Design review of the part shown in the three views and the two pictorial views. Dimensions are in mm from the part's minimum x, y and z. A direction names the side the tool comes from. Round coordinates to 2 decimals unless told otherwise and drop trailing zeros. Loops run counter-clockwise (first coordinate to the right, second up) from the corner with the lowest first, then second, coordinate; pieces in that order, holes last.
1. Clearance check with flat-ended pins moving along their axes: pin 1 Ø17.5 at (x, y) = (31, 45) entering from +Z; pin 2 Ø12 at (x, z) = (50, 108) entering from +Y; pin 3 Ø3 at (x, z) = (20, 16.5) entering from +Y. State where each tip first meets the part, or that it passes through.
2. Tool access review of the marked faces 1, 2, 3 and 4: name each direction out of +Z, -Z, +X, -X, +Y, -Y from which nothing blocks a thin tool from reaching the whole face with its end or side.
3. To check wall thickness, follow line 1 along Y through (x, z) = (49.5, 134) (1 decimal); line 2 along Y through (x, z) = (37, 35.5); line 3 along Y through (x, z) = (48.5, 8.5). State the ranges of each line that lie inside material, in increasing order.
4. Consider section A-A on x = 34. State the section outline as (y, z) points, then the cut area to 3 significant figures.
5. Draft analysis for pull direction Z (two halves, no side actions). For the marked faces 5, 6 and 7, state which applies: released by +Z, released by -Z, zero draft, split by the parting line, or undercut.
6. Consider section C-C on z = 28. State the section outline as (x, y) points, then the cut area to 3 significant figures.
7. Consider section D-D on x = 54. State the section outline as (y, z) points, then the cut area to 3 significant figures.
8. Consider section B-B on y = 37.5. State the section outline as (x, z) points, then the cut area to 3 significant figures.
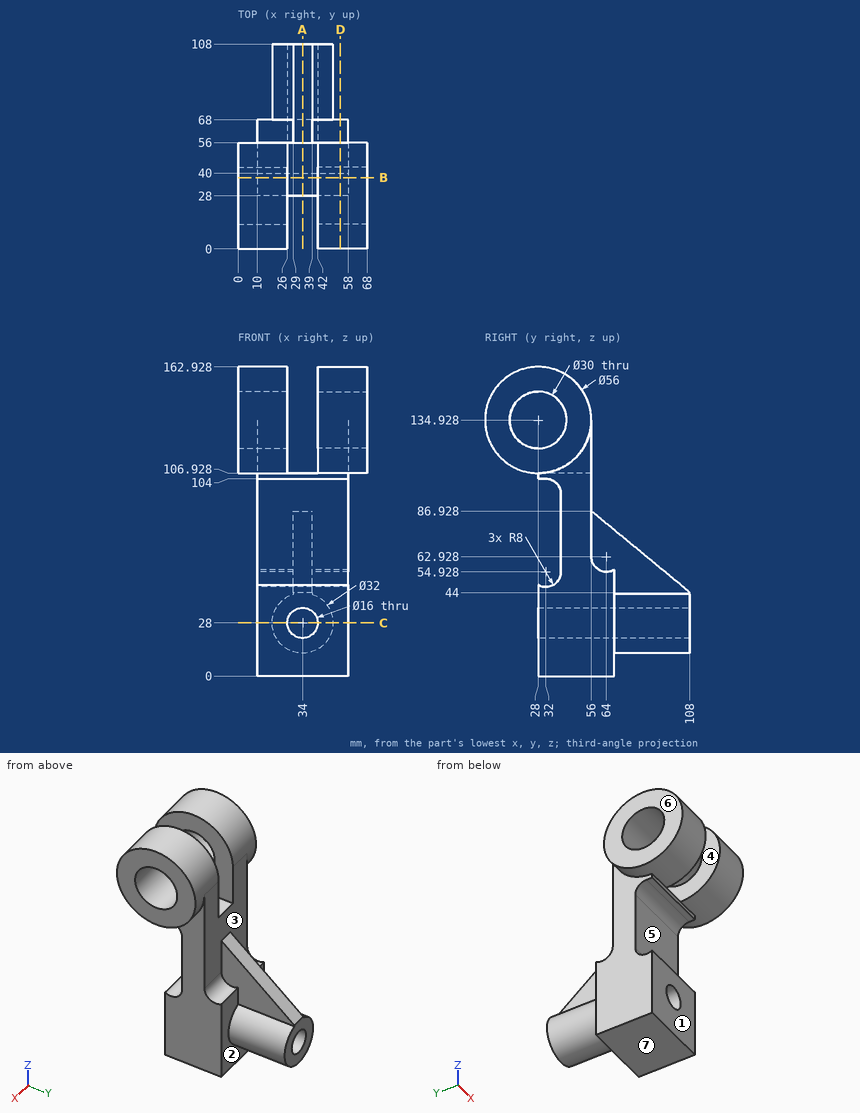
Resolved:
1. pin 1: stops at z = 161.15
1. pin 2: stops at y = 56
1. pin 3: stops at y = 68
2. face 1: -Z, +X, -X, -Y
2. face 2: +Y
2. face 3: +Z, +Y
2. face 4: +Z, +Y, -Y
3. line 1: y = 0 to 13, 43 to 56
3. line 2: y = 28 to 108
3. line 3: y = 28 to 68
4. outline: (28, 0) - (68, 0) - (68, 12) - (108, 12) - (108, 20) - (28, 20) - close; (28, 36) - (108, 36) - (108, 44) - (56, 86.93) - (56, 106.93) - (28, 106.93) - (28, 104) - (32, 104) arc R8 cw to (40, 96) - (40, 54.93) arc R8 cw to (28, 48) - close
4. area: 3,980 mm2
5. face 5: undercut
5. face 6: zero draft
5. face 7: released by -Z
6. outline: (10, 28) - (26, 28) - (26, 108) - (18, 108) - (18, 68) - (10, 68) - close; (42, 28) - (58, 28) - (58, 68) - (50, 68) - (50, 108) - (42, 108) - close
6. area: 1,920 mm2
7. outline: (28, 0) - (68, 0) - (68, 56) arc R8 cw to (56, 62.93) - (56, 134.93) arc R28 ccw (long way) to (28, 106.93) - (28, 104) - (32, 104) arc R8 cw to (40, 96) - (40, 54.93) arc R8 cw to (28, 48) - close; hole circle Ø30 at (28, 134.93)
7. area: 4,940 mm2
8. outline: (0, 108.59) - (10, 108.59) - (10, 101.81) - (58, 101.81) - (58, 108.59) - (68, 108.59) - (68, 123.32) - (42, 123.32) - (42, 106.93) - (26, 106.93) - (26, 123.32) - (0, 123.32) - close; (0, 146.54) - (26, 146.54) - (26, 161.27) - (0, 161.27) - close; (10, 0) - (58, 0) - (58, 49.12) - (10, 49.12) - close; (42, 146.54) - (68, 146.54) - (68, 161.27) - (42, 161.27) - close; hole circle Ø16 at (34, 28)
8. area: 3,990 mm2
